CAD build for the part. Positions are in the model's coordinates, mm. Round coordinates to 2 decimals unless told otherwise and drop trailing zeros. Loops run counter-clockwise (first coordinate to the right, second up) from the corner with the lowest first, then second, coordinate; pieces in that order, holes last. Notation, with made-up numbers: M 67,16 L 73,16 A30 cw 73,40 Z; hole C 77,-11 d2. An arc over 180 degrees is marked long. One line per item, written item: value. Start each with the question number.
from build123d import *

# Parameters (mm, degrees)
SKETCH1_R               = 1.85
BOSS_EXTRUDE1_DEPTH     = 230
SKETCH2_R               = 2.5
BOSS_EXTRUDE2_DEPTH     = 30
CHAMFER1_SIZE           = 1.8
CHAMFER1_SIZE2          = 20
CUT_EXTRUDE1_DEPTH      = 10
CUT_EXTRUDE1_DEPTH_BACK = 10
SKETCH_3_2_R            = 1


with BuildPart() as part:
    # Sketch1 → Boss-Extrude1 (new body)
    with BuildSketch(Plane.XY):
        Circle(SKETCH1_R)
    extrude(amount=BOSS_EXTRUDE1_DEPTH)

    # Sketch2 → Boss-Extrude2 (add)
    with BuildSketch(Plane.XY.offset(230)):
        Circle(SKETCH2_R)
    extrude(amount=BOSS_EXTRUDE2_DEPTH)

    # Chamfer1
    chamfer1_edges = [part.edges().sort_by_distance(p)[0] for p in [
        (-1.85, 0, 0),
    ]]
    chamfer1_side = [part.faces().sort_by_distance(p)[0] for p in [
        (0, 0, 0),
    ]]
    chamfer(chamfer1_edges, length=CHAMFER1_SIZE, length2=CHAMFER1_SIZE2, reference=chamfer1_side[0])

    # Sketch 3_2 → Cut-Extrude1 (cut, two sides: drawn at the far end of the back side and taken through both)
    with BuildSketch(Plane(origin=(0, 0, 0), x_dir=(1, 0, 0), z_dir=(0, 1, 0)).offset(-CUT_EXTRUDE1_DEPTH_BACK)):
        with Locations(Location((0, -250, 0), (0, 0, 90))):
            Circle(SKETCH_3_2_R)
    extrude(amount=CUT_EXTRUDE1_DEPTH + CUT_EXTRUDE1_DEPTH_BACK, mode=Mode.SUBTRACT)


solid = part.part
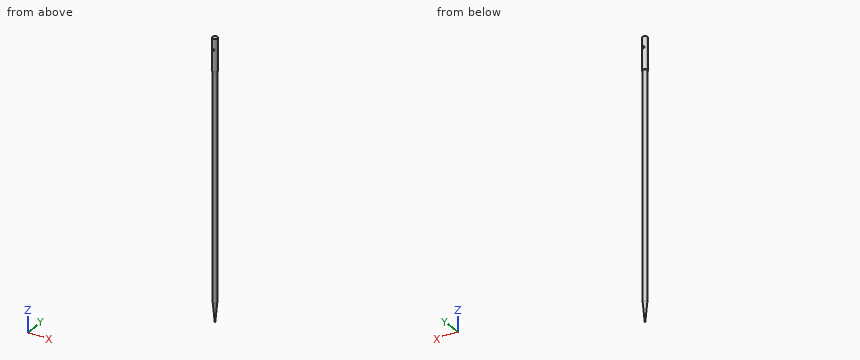
(1) Slice it at A-A, the plane z = 184. List the corners of the cut face in (x, y), and give its area (3 significant figures).
(2) Probe L1, parallel to Z at x = 0.15, y = -2; L2, parallel to X at y = 0.2, z = 31; L3, parallel to Y at x = -0.4, z = 53.5. List the from-to ranges inside material, lowest first.
(3) Flat gauge pin, fed straight in: P1, Ø2, axis at x = 1, z = 137, coming from the -Y side. Where does the tip first touch, or does it go through?
Check result:
1. outline: C 0,0 d3.7
1. area: 10.8 mm^2
2. L1: z = 230 to 249.01, 250.99 to 260
2. L2: x = -1.84 to 1.84
2. L3: y = -1.81 to 1.81
3. P1: stops at y = -1.85
